```python
from build123d import *
from OCP.BRepFilletAPI import BRepFilletAPI_MakeChamfer

# Parameters (mm, degrees)
EXTRUDE_1_DEPTH          = 1160
CUT_EXTRUDE_1_DEPTH      = 1164.587555795
CUT_EXTRUDE_1_DEPTH_BACK = 1164.587555795
CHAMFER_1_SIZE           = 6
CHAMFER_1_SIZE2          = 6.742931709


with BuildPart() as part:
    # 草图1 → 凸台-拉伸1 (new, symmetric)
    with BuildSketch(Plane.XY):
        Polygon((44, 80), (-44, 80), (-44, 76), (-3, 72), (-3, -72), (-44, -76), (-44, -80), (44, -80), (44, -76), (3, -72), (3, 72), (44, 76), align=None)
    extrude(amount=EXTRUDE_1_DEPTH, both=True)

    # 草图3 → 切除-拉伸1 (cut, two sides: drawn at the far end of the back side and taken through both)
    with BuildSketch(Plane(origin=(0, 0, 0), x_dir=(0, 0, -1), z_dir=(1, 0, 0)).offset(-CUT_EXTRUDE_1_DEPTH_BACK)):
        Polygon((-1160, 66), (-1103, 72), (-1103, 80), (-1160, 80), align=None)
        Polygon((1160, 80), (1160, 66), (1103, 72), (1103, 80), align=None)
        Polygon((1160, -66), (1103, -72), (1103, -80), (1160, -80), align=None)
        Polygon((-1160, -80), (-1160, -66), (-1103, -72), (-1103, -80), align=None)
    extrude(amount=CUT_EXTRUDE_1_DEPTH + CUT_EXTRUDE_1_DEPTH_BACK, mode=Mode.SUBTRACT)

    # 倒角1: one chamfer whose edges measure the first distance from different faces: ONE call of the kernel's chamfer builder (chamfer() names one face for all edges)
    chamfer_1_edges_1 = [part.edges().sort_by_distance(p)[0] for p in [
        (0, 66, -1160),
        (0, -66, -1160),
    ]]
    chamfer_1_side_1 = [part.faces().sort_by_distance(p)[0] for p in [
        (0, 0, -1160),
    ]]
    chamfer_1_edges_2 = [part.edges().sort_by_distance(p)[0] for p in [
        (0, 66, 1160),
    ]]
    chamfer_1_side_2 = [part.faces().sort_by_distance(p)[0] for p in [
        (0, 69, 1131.5),
    ]]
    chamfer_1_edges_3 = [part.edges().sort_by_distance(p)[0] for p in [
        (0, -66, 1160),
    ]]
    chamfer_1_side_3 = [part.faces().sort_by_distance(p)[0] for p in [
        (0, -69, 1131.5),
    ]]
    chamfer_1 = BRepFilletAPI_MakeChamfer(part.part.solid().wrapped)
    for e in chamfer_1_edges_1:
        chamfer_1.Add(CHAMFER_1_SIZE, CHAMFER_1_SIZE2, e.wrapped, chamfer_1_side_1[0].wrapped)  # the first distance lies on this face
    for e in chamfer_1_edges_2:
        chamfer_1.Add(CHAMFER_1_SIZE, CHAMFER_1_SIZE2, e.wrapped, chamfer_1_side_2[0].wrapped)  # the first distance lies on this face
    for e in chamfer_1_edges_3:
        chamfer_1.Add(CHAMFER_1_SIZE, CHAMFER_1_SIZE2, e.wrapped, chamfer_1_side_3[0].wrapped)  # the first distance lies on this face
    add(Compound.cast(chamfer_1.Shape()), mode=Mode.REPLACE)


solid = part.part
```
For this review, take the finished solid that the model builds, in its own axes (mm). A direction names the side the tool comes from. Coordinates: 2 decimals unless noted, no trailing zeros. Write each loop counter-clockwise with the first axis right and the second up, starting at its lowest first coordinate (ties: lowest second). Pieces come first, ordered by that corner, then holes. Notation, with made-up numbers: (72.5, 6) - (81.5, 6) arc R33 cw to (81.5, 34) - close; hole circle Ø3 at (48.25, -12.5). An arc over 180 degrees is marked (long way). Answer in a Markdown table with one row per item. Add a question column.
Q1. For P1, Ø8, axis at y = -25.5, z = -229, coming from the +X side; P2, Ø9, axis at x = -20.5, y = 75.5, coming from the -Z side; P3, Ø4, axis at x = -13.5, y = -75, coming from the +Z side, all flat-tipped, find the tip position at first contact; note any pin that passes through.
Q2. We need section A-A, the plane z = -356. State the section outline as (x, y) points.
Q3. We need section C-C, the plane y = 9. State the section outline as (x, z) points.
Q4. Tool access review of faces 4 (the flat face through (-3, 1, 16)), 5 (the flat face through (23.79, -74.03, 15.44)): name each direction out of +Z, -Z, +X, -X, +Y, -Y from which nothing blocks a thin tool from reaching the whole face with its end or side.
Q5. For probe 1 along Y at (x, z) = (40, -925); probe 2 along Y at (x, z) = (19, -172.5); probe 3 along X at (y, z) = (-61, 373.5), list the stretches that pass through material, from the lowest coordinate up.
Q6. Draft analysis for pull direction Y (two halves, no side actions). For faces 1 (the flat face through (1, 80, 15)), 2 (the flat face through (-23.21, -73.97, 15.44)), 3 (the flat face through (-1, -80, 15)), state which applies: +Y half, -Y half, draft (parallel to the pull), parting line (faces both ways), or undercut.
Q7. We need section B-B, the plane x = 27.5. State the section outline as (y, z) points.
Answer list:
| question | item | result |
|---|---|---|
| 1 | P1 | stops at x = 3 |
| 1 | P2 | stops at z = -1103 |
| 1 | P3 | stops at z = 1103 |
| 2 | outline | (-44, -80) - (44, -80) - (44, -76) - (3, -72) - (3, 72) - (44, 76) - (44, 80) - (-44, 80) - (-44, 76) - (-3, 72) - (-3, -72) - (-44, -76) - close |
| 3 | outline | (-3, -1160) - (3, -1160) - (3, 1160) - (-3, 1160) - close |
| 4 | face 4 | +Z, -Z, -X |
| 4 | face 5 | +Z, -Z, +X |
| 5 | probe 1 | y = -80 to -75.61, 75.61 to 80 |
| 5 | probe 2 | y = -80 to -73.56, 73.56 to 80 |
| 5 | probe 3 | x = -3 to 3 |
| 6 | face 1 | +Y half |
| 6 | face 2 | undercut |
| 6 | face 3 | -Y half |
| 7 | outline | (-80, -1103) - (-74.39, -1103) - (-74.39, 1103) - (-80, 1103) - close; (74.39, -1103) - (80, -1103) - (80, 1103) - (74.39, 1103) - close |
